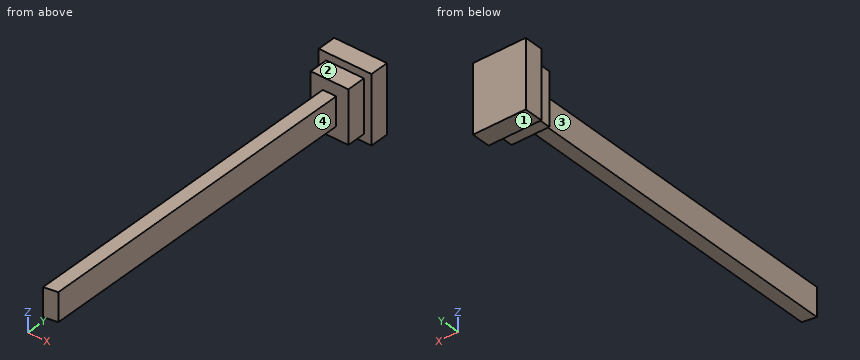
```python
from build123d import *

# Parameters (mm, degrees)
SKETCH1_W           = 1.78
SKETCH1_H           = 3.78
BOSS_EXTRUDE1_DEPTH = 45
CUT_EXTRUDE1_DEPTH  = 46.167250304
SKETCH3_W           = 5
SKETCH3_H           = 7
BOSS_EXTRUDE2_DEPTH = 2.5
SKETCH4_W           = 7
SKETCH4_H           = 9
BOSS_EXTRUDE3_DEPTH = 2.5


with BuildPart() as part:
    # Sketch1 → Boss-Extrude1 (new body)
    with BuildSketch(Plane(origin=(0, 0, 0), x_dir=(1, 0, 0), z_dir=(0, 1, 0))):
        Rectangle(SKETCH1_W, SKETCH1_H)
    extrude(amount=BOSS_EXTRUDE1_DEPTH)

    # Sketch2 → Cut-Extrude1 (cut, through all)
    with BuildSketch(Plane.XY.offset(1.89)):
        Polygon((-0.89, 0), (0.89, 0), (0.89, 0.313862026), align=None)
    extrude(amount=-CUT_EXTRUDE1_DEPTH, mode=Mode.SUBTRACT)

    # Sketch3 → Boss-Extrude2 (add)
    with BuildSketch(Plane(origin=(0, 45, 0), x_dir=(1, 0, 0), z_dir=(0, 1, 0))):
        Rectangle(SKETCH3_W, SKETCH3_H)
    extrude(amount=BOSS_EXTRUDE2_DEPTH)

    # Sketch4 → Boss-Extrude3 (add)
    with BuildSketch(Plane(origin=(0, 47.5, 0), x_dir=(1, 0, 0), z_dir=(0, 1, 0))):
        Rectangle(SKETCH4_W, SKETCH4_H)
    extrude(amount=BOSS_EXTRUDE3_DEPTH)


solid = part.part
```
The model under review builds one solid part; all positions refer to its coordinate system, in mm. Face numbers are marked on the shaded views. A direction names the side the tool comes from. Give positions to 0.01 mm unless a question says otherwise; leave off trailing zeros. Write each loop counter-clockwise with the first axis right and the second up, starting at its lowest first coordinate (ties: lowest second). Pieces come first, ordered by that corner, then holes. Notation, with made-up numbers: M 31,-16.75 L 57,-16.75 A20 cw 57,-7.75 Z; hole C 86.5,14 d6. An arc over 180 degrees is marked long. Write each question's results on one line, items separated by ' | '. Start each with the question number.
1. Insertion check: pin 1 Ø1.1 at (y, z) = (25, -0.5) entering from -X; pin 2 Ø2 at (x, y) = (-0.5, 17) entering from +Z; pin 3 Ø1.1 at (y, z) = (13.5, 0.5) entering from +X. Each pin has a flat end and moves straight along its axis. Give the tip position at first contact, or say it passes through.
2. For probe 1 along Z at (x, y) = (0.75, 15); probe 2 along X at (y, z) = (6, 0.5); probe 3 along Y at (x, z) = (0.75, -3.25), list the stretches that pass through material, from the lowest coordinate up. Write a range as [from, to].
3. We need section B-B (x = 1.5). Write out the cut boundary in (y, z), and give its area (3 significant figures).
4. We need section C-C (y = 7). Write out the cut boundary in (x, z).
5. We need section D-D (z = 2.5). Write out the cut boundary in (x, y), and give its area (3 significant figures).
6. We need section A-A (z = -1.25). Write out the cut boundary in (x, y).
7. For the marked faces 1, 2, 3 and 4, list the 3-axis set-ups (+Z, -Z, +X, -X, +Y, -Y) from which the entire face can be reached by the end or side of a thin tool; tool diameter is ignored.
Results found:
1) pin 1: stops at x = -0.89 | pin 2: stops at z = 1.89 | pin 3: stops at x = 0.89
2) probe 1: z = [-1.89, 1.89] | probe 2: x = [-0.89, 0.89] | probe 3: y = [45, 50]
3) outline: M 45,-3.5 L 47.5,-3.5 L 47.5,-4.5 L 50,-4.5 L 50,4.5 L 47.5,4.5 L 47.5,3.5 L 45,3.5 Z | area: 40.0 mm^2
4) outline: M -0.89,-1.89 L 0.89,-1.89 L 0.89,1.89 L -0.89,1.89 Z
5) outline: M -3.5,47.5 L -2.5,47.5 L -2.5,45 L 2.5,45 L 2.5,47.5 L 3.5,47.5 L 3.5,50 L -3.5,50 Z | area: 30.0 mm^2
6) outline: M -3.5,47.5 L -2.5,47.5 L -2.5,45 L -0.89,45 L -0.89,0 L 0.89,0.31 L 0.89,45 L 2.5,45 L 2.5,47.5 L 3.5,47.5 L 3.5,50 L -3.5,50 Z
7) face 1: -Z, +X, -X, +Y, -Y | face 2: +Z, +X, -X, -Y | face 3: +Z, -Z, -X, -Y | face 4: +Z, -Z, +X, -Y
